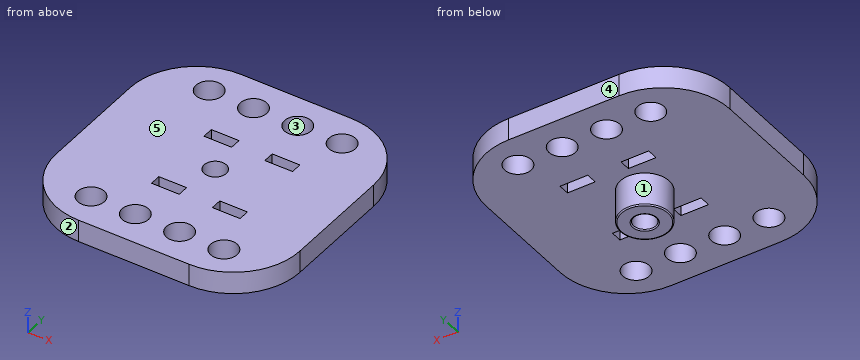
```python
from build123d import *

# Parameters (mm, degrees)
SKETCH_1_R          = 6
SKETCH_1_W          = 12.5
SKETCH_1_H          = 5
EXTRUDE_1_DEPTH     = 10
SKETCH_2_R          = 11
EXTRUDE_2_DEPTH     = 15
SKETCH_3_R          = 5
CUT_EXTRUDE_1_DEPTH = 25
FILLET_1_R          = 0.5
FILLET_2_R          = 0.5


with BuildPart() as part:
    # 草图1 → 凸台-拉伸1 (new body)
    with BuildSketch(Plane.XY):
        with BuildLine():
            Line((-25.422431237, 54.841573229), (24.577568763, 54.841573229))
            ThreePointArc((24.577568763, 54.841573229), (45.790772199, 46.054776665), (54.577568763, 24.841573229))
            Line((54.577568763, 24.841573229), (54.577568763, -25.158426771))
            ThreePointArc((54.577568763, -25.158426771), (45.790772199, -46.371630206), (24.577568763, -55.158426771))
            Line((24.577568763, -55.158426771), (-25.422431237, -55.158426771))
            ThreePointArc((-25.422431237, -55.158426771), (-46.635634673, -46.371630206), (-55.422431237, -25.158426771))
            Line((-55.422431237, -25.158426771), (-55.422431237, 24.841573229))
            ThreePointArc((-55.422431237, 24.841573229), (-46.635634673, 46.054776665), (-25.422431237, 54.841573229))
        make_face()
        with Locations((-29.718021333, 39.841573229)):
            Circle(SKETCH_1_R, mode=Mode.SUBTRACT)
        with Locations((-9.718021333, 39.841573229)):
            Circle(SKETCH_1_R, mode=Mode.SUBTRACT)
        with Locations((10.281978667, 39.841573229)):
            Circle(SKETCH_1_R, mode=Mode.SUBTRACT)
        with Locations((30.281978667, 39.841573229)):
            Circle(SKETCH_1_R, mode=Mode.SUBTRACT)
        with Locations((30.281978667, -40.158426771)):
            Circle(SKETCH_1_R, mode=Mode.SUBTRACT)
        with Locations((10.281978667, -40.158426771)):
            Circle(SKETCH_1_R, mode=Mode.SUBTRACT)
        with Locations((-9.718021333, -40.158426771)):
            Circle(SKETCH_1_R, mode=Mode.SUBTRACT)
        with Locations((-29.718021333, -40.158426771)):
            Circle(SKETCH_1_R, mode=Mode.SUBTRACT)
        with Locations((18.327568763, 17.341573229)):
            Rectangle(SKETCH_1_W, SKETCH_1_H, mode=Mode.SUBTRACT)
        with Locations((18.327568763, -18.158426771)):
            Rectangle(SKETCH_1_W, SKETCH_1_H, mode=Mode.SUBTRACT)
        with Locations((-9.172431237, -18.158426771)):
            Rectangle(SKETCH_1_W, SKETCH_1_H, mode=Mode.SUBTRACT)
        with Locations((-9.172431237, 17.341573229)):
            Rectangle(SKETCH_1_W, SKETCH_1_H, mode=Mode.SUBTRACT)
    extrude(amount=EXTRUDE_1_DEPTH)

    # 草图2 → 凸台-拉伸2 (add)
    with BuildSketch(Plane(origin=(0, 0, 0), x_dir=(-1, 0, 0), z_dir=(0, 0, -1))):
        with Locations(Location((0.422431237, 0, 0), (0, 0, 180))):
            Circle(SKETCH_2_R)
    extrude(amount=EXTRUDE_2_DEPTH)

    # 草图3 → 切除-拉伸1 (cut)
    with BuildSketch(Plane(origin=(0, 0, -15), x_dir=(-1, 0, 0), z_dir=(0, 0, -1))):
        with Locations((0.422431237, 0)):
            Circle(SKETCH_3_R)
    extrude(amount=-CUT_EXTRUDE_1_DEPTH, mode=Mode.SUBTRACT)

    # 圆角1
    fillet_1_edges = [part.edges().sort_by_distance(p)[0] for p in [
        (4.577568763, 0, -15),
    ]]
    fillet(fillet_1_edges, radius=FILLET_1_R)

    # 圆角2
    fillet_2_edges = [part.edges().sort_by_distance(p)[0] for p in [
        (-11.422431237, 0, -15),
    ]]
    fillet(fillet_2_edges, radius=FILLET_2_R)


solid = part.part
```
Verification items for the finished model (mm, model axes). Face numbers are marked on the shaded views. A direction names the side the tool comes from. Coordinates: 2 decimals unless noted, no trailing zeros. Order: outer loops, then holes, each group sorted by start corner. A loop starts at its lowest first (then second) coordinate and runs counter-clockwise, first axis right, second up. Notation, with made-up numbers: (14, 4.5) -> (34, 4.5) arc R16 cw to (34, 35.5) -> close; hole circle Ø9 at (5.25, 22). An arc over 180 degrees is marked (long way). Answer as CSV lines item,"result". Start each with the question number.
1) Gauge pin test, flat ends, axial feed: pin 1 Ø14 at (x, y) = (10.28, 39.84) entering from -Z; pin 2 Ø1 at (y, z) = (42.5, 2) entering from +X; pin 3 Ø2 at (y, z) = (-8.5, -9.5) entering from -X; pin 4 Ø2 at (y, z) = (12, -0.5) entering from +X. Record the tip position at first contact, or that the pin passes through.
2) Cross-section at D-D, the plane y = -35.5. Record the boundary of the cut face in (x, z).
3) Release check for a two-part mould opening along Y. For the marked faces 3, 4 and 5 record: released by +Y, released by -Y, zero draft, split by the parting line, or undercut.
4) Set-up check for the marked faces 1 and 2: record each of +Z, -Z, +X, -X, +Y, -Y from which the full face is reachable in a straight line by a thin tool's end or side.
5) Material ranges on L1, parallel to Y at x = 10, z = 3.5; L2, parallel to X at y = 40, z = 3; L3, parallel to Y at x = -34.5, z = 1.75, recorded low to high. Write a range as [from, to].
6) Cross-section at B-B, the plane y = 0. Record the boundary of the cut face in (x, z).
7) Cross-section at A-A, the plane x = -13.5. Record the boundary of the cut face in (y, z).
8) Cross-section at C-C, the plane z = -5.5. Record the boundary of the cut face in (x, y), then the cut area to 3 significant figures.
Conclusion:
1,pin 1,"stops at z = 0"
1,pin 2,"stops at x = 49.19"
1,pin 3,"stops at x = -8.47"
1,pin 4,"stops at x = 54.58"
2,outline,"(-53.58, 0) -> (-33.5, 0) -> (-33.5, 10) -> (-53.58, 10) -> close; (-25.94, 0) -> (-13.5, 0) -> (-13.5, 10) -> (-25.94, 10) -> close; (-5.94, 0) -> (6.5, 0) -> (6.5, 10) -> (-5.94, 10) -> close; (14.06, 0) -> (26.5, 0) -> (26.5, 10) -> (14.06, 10) -> close; (34.06, 0) -> (52.74, 0) -> (52.74, 10) -> (34.06, 10) -> close"
3,face 3,"undercut"
3,face 4,"released by +Y"
3,face 5,"zero draft"
4,face 1,"-Z"
4,face 2,"+Z, -Z, -X, -Y"
5,L1,"y = [-55.16, -46.15], [-34.17, 33.85], [45.83, 54.84]"
5,L2,"x = [-51.31, -35.72], [-23.72, -15.72], [-3.72, 4.28], [16.28, 24.28], [36.28, 50.47]"
5,L3,"y = [-53.75, -43.78], [-36.53, 36.22], [43.47, 53.44]"
6,outline,"(-55.42, 0) -> (-11.42, 0) -> (-11.42, -14.5) arc R0.5 ccw to (-10.92, -15) -> (-5.92, -15) arc R0.5 ccw to (-5.42, -14.5) -> (-5.42, 10) -> (-55.42, 10) -> close; (4.58, -14.5) arc R0.5 ccw to (5.08, -15) -> (10.08, -15) arc R0.5 ccw to (10.58, -14.5) -> (10.58, 0) -> (54.58, 0) -> (54.58, 10) -> (4.58, 10) -> close"
7,outline,"(-55.16, 0) -> (-44.82, 0) -> (-44.82, 10) -> (-55.16, 10) -> close; (-35.5, 0) -> (-20.66, 0) -> (-20.66, 10) -> (-35.5, 10) -> close; (-15.66, 0) -> (14.84, 0) -> (14.84, 10) -> (-15.66, 10) -> close; (19.84, 0) -> (35.18, 0) -> (35.18, 10) -> (19.84, 10) -> close; (44.5, 0) -> (54.84, 0) -> (54.84, 10) -> (44.5, 10) -> close"
8,outline,"circle Ø22 at (-0.42, 0); hole circle Ø10 at (-0.42, 0)"
8,area,"302 mm²"
